Geometry check sheet. Reference: the model listing, model coordinates, mm. Face numbers are marked on the shaded views. A direction names the side the tool comes from. Round coordinates to 2 decimals unless told otherwise and drop trailing zeros. Order: outer loops, then holes, each group sorted by start corner. A loop starts at its lowest first (then second) coordinate and runs counter-clockwise, first axis right, second up. Notation, with made-up numbers: (56.5, -30.5) - (90.5, -30.5) arc R15 ccw to (90.5, -3.5) - close; hole circle Ø6 at (42, -8.75). An arc over 180 degrees is marked (long way). Use a Markdown table: item, result. Add a question column.
(1) Section check C-C on x = -2.5. Record the boundary of the cut face in (y, z).
(2) Gauge pin test, flat ends, axial feed: P1, Ø6, axis at x = -11, z = 21.5, coming from the +Y side; P2, Ø10, axis at x = -4.5, y = 25, coming from the -Z side; P3, Ø14.5, axis at y = 9, z = -1.5, coming from the +X side. Record the tip position at first contact, or that the pin passes through.
(3) Thickness scan on line 1 along Y through (x, z) = (-11.5, 24); line 2 along Z through (x, y) = (-18, 0); line 3 along X through (y, z) = (-26, 19). Record the ranges inside material, lowest first. Write a range as [from, to].
(4) Section check D-D on x = -21.75. Record the boundary of the cut face in (y, z).
(5) Mould release check, pull along Y, two halves, no side actions. Record for the marked faces 1, 2 and 3: released by +Y, released by -Y, zero draft, split by the parting line, or undercut.
(6) Access from +Z, -Z, +X, -X, +Y, -Y to the whole of each face (thin tool, end or side, straight path). Record for the marked faces 4, 5 and 6.
(7) Section check A-A on z = -23. Record the boundary of the cut face in (x, y), then the cut area to 3 significant figures.
```python
from build123d import *

# Parameters (mm, degrees)
CBORE_SOCKET_HEAD_CAP_SCREW1_D           = 6.6
CBORE_SOCKET_HEAD_CAP_SCREW1_CBORE_D     = 11
CBORE_SOCKET_HEAD_CAP_SCREW1_CBORE_DEPTH = 6.5
TAPPED_HOLE1_D                           = 2.5
TAPPED_HOLE1_DEPTH                       = 8.5
TAPPED_HOLE1_TIP                         = 0.751075774
CHAMFER1_SIZE                            = 0.5


with BuildPart() as part:
    # Sketch1 → Revolve1 (revolve)
    with BuildSketch(Plane.XY):
        Polygon((0, 24), (-6, 24), (-6, 16), (-26, 16), (-26, 14), (-29, 14), (-29, 25), (-12, 25), (-12, 37.5), (0, 37.5), align=None)
    revolve(axis=Axis((0, 0, 0), (-1, 0, 0)))

    # CBORE Socket Head Cap Screw1 (through all)
    with Locations(Plane(origin=(0, 0, 0), x_dir=(0, 0, -1), z_dir=(1, 0, 0))):
        with Locations((-21.920310217, 21.920310217), (21.920310217, 21.920310217), (21.920310217, -21.920310217), (-21.920310217, -21.920310217)):
            CounterBoreHole(CBORE_SOCKET_HEAD_CAP_SCREW1_D / 2, CBORE_SOCKET_HEAD_CAP_SCREW1_CBORE_D / 2, CBORE_SOCKET_HEAD_CAP_SCREW1_CBORE_DEPTH)

    # Tapped Hole1
    with Locations(Plane(origin=(-6, 0, 0), x_dir=(0, 0, -1), z_dir=(1, 0, 0))):
        with Locations((0, 20), (-20, 0), (0, -20), (20, 0)):
            Hole(TAPPED_HOLE1_D / 2, depth=TAPPED_HOLE1_DEPTH)
            with Locations((0, 0, -(TAPPED_HOLE1_DEPTH + TAPPED_HOLE1_TIP / 2))):  # 118° drill point
                Cone(0, TAPPED_HOLE1_D / 2, TAPPED_HOLE1_TIP, mode=Mode.SUBTRACT)

    # Chamfer1
    chamfer1_edges = [part.edges().sort_by_distance(p)[0] for p in [
        (-6, -16, 0),
    ]]
    chamfer(chamfer1_edges, length=CHAMFER1_SIZE)


solid = part.part
```
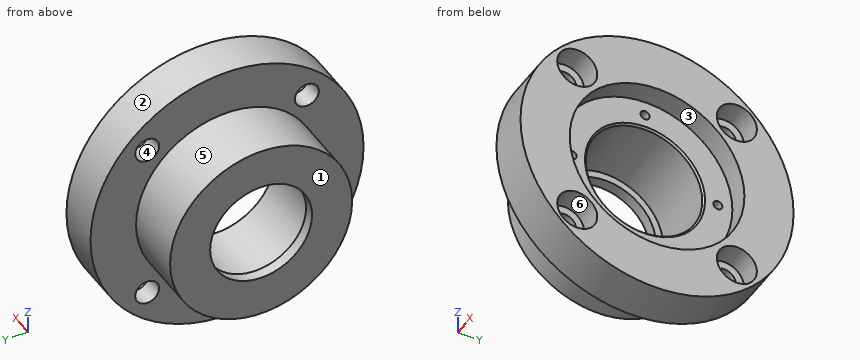
Check sheet entries:
| question | item | result |
|---|---|---|
| 1 | outline | circle Ø75 at (0, 0); hole circle Ø11 at (-21.92, -21.92); hole circle Ø11 at (-21.92, 21.92); hole circle Ø48 at (0, 0); hole circle Ø11 at (21.92, -21.92); hole circle Ø11 at (21.92, 21.92) |
| 2 | P1 | stops at y = 32.62 |
| 2 | P2 | stops at z = -31.72 |
| 2 | P3 | stops at x = -6.13 |
| 3 | line 1 | y = [-28.81, -24.48], [-19.36, 19.36], [24.48, 28.81] |
| 3 | line 2 | z = [-25, -16], [16, 25] |
| 3 | line 3 | x = [-12, -6.5] |
| 4 | outline | circle Ø50 at (0, 0); hole circle Ø32 at (0, 0) |
| 5 | face 1 | zero draft |
| 5 | face 2 | split by the parting line |
| 5 | face 3 | undercut |
| 6 | face 4 | +X, -X |
| 6 | face 5 | -X |
| 6 | face 6 | +X |
| 7 | outline | (-29, -9.8) - (-12, -9.8) - (-12, -18.8) - (-6.5, -18.8) - (-6.5, -16.53) - (0, -16.53) - (0, -6.86) - (-6, -6.86) - (-6, 6.86) - (0, 6.86) - (0, 16.53) - (-6.5, 16.53) - (-6.5, 18.8) - (-12, 18.8) - (-12, 9.8) - (-29, 9.8) - close; (-12, -29.62) - (0, -29.62) - (0, -27.31) - (-6.5, -27.31) - (-6.5, -25.04) - (-12, -25.04) - close; (-12, 25.04) - (-6.5, 25.04) - (-6.5, 27.31) - (0, 27.31) - (0, 29.62) - (-12, 29.62) - close |
| 7 | area | 753 mm2 |
